Could you check a few things on this model? Use its own coordinates, in mm. A direction names the side the tool comes from. Coordinates: 2 decimals unless noted, no trailing zeros. Order: outer loops, then holes, each group sorted by start corner. A loop starts at its lowest first (then second) coordinate and runs counter-clockwise, first axis right, second up. Notation, with made-up numbers: M 54.5,84 L 82.5,84 A26 cw 82.5,117 Z; hole C 1,-26 d8. An arc over 180 degrees is marked long. Put each result on its own line as item: value. Start each with the question number.
```python
from build123d import *
from build123d.topology import SkipClean

# Parameters (mm, degrees)
CUT_EXTRUDE1_DEPTH      = 13.124356
CUT_EXTRUDE1_DEPTH_BACK = 13.124356
SKETCH4_R               = 3
CUT_EXTRUDE2_DEPTH      = 16.556349
CHAMFER1_SIZE           = 0.4
FILLET1_R               = 5


with BuildPart() as part:
    # Sketch1 → Boss-Revolve (revolve)
    with BuildSketch(Plane.XY):
        with BuildLine():
            Line((-7, 0), (7, 0))
            ThreePointArc((7, 0), (0, 7), (-7, 0))
        make_face()
    revolve(axis=Axis((-13.286843, 0, 0), (1, 0, 0)))

    # Sketch2 → Cut-Extrude1 (cut, two sides: drawn at the far end of the back side and taken through both)
    with SkipClean():  # the faces are left unmerged after this step: merging them gives an invalid solid
        with BuildSketch(Plane(origin=(0, 0, 0), x_dir=(0, 0, -1), z_dir=(1, 0, 0)).offset(-CUT_EXTRUDE1_DEPTH_BACK)):
            with BuildLine():
                Line((-5, 4.898979), (-5, -4.898979))
                ThreePointArc((-5, -4.898979), (-7, 0), (-5, 4.898979))
            make_face()
            with BuildLine():
                Line((5, 4.898979), (5, -4.898979))
                ThreePointArc((5, -4.898979), (7, 0), (5, 4.898979))
            make_face()
        extrude(amount=CUT_EXTRUDE1_DEPTH + CUT_EXTRUDE1_DEPTH_BACK, mode=Mode.SUBTRACT)

    # Sketch4 → Cut-Extrude2 (cut, through all)
    with SkipClean():  # the faces are left unmerged after this step: merging them gives an invalid solid
        with BuildSketch(Plane.XY.offset(5)):
            Circle(SKETCH4_R)
        extrude(amount=-CUT_EXTRUDE2_DEPTH, mode=Mode.SUBTRACT)

    # Sketch5 → Boss-Revolve1 (revolve)
    with SkipClean():  # the faces are left unmerged after this step: merging them gives an invalid solid
        with BuildSketch(Plane.XY, mode=Mode.PRIVATE) as boss_revolve1_sk:
            Polygon((3.469445, 3.45875), (3.469445, 0), (50, 0), (50, 4), (28, 4), (27.062528, 3.45875), align=None)
        revolve(boss_revolve1_sk.sketch.rotate(Axis((0, 0, 0), (1, 0, 0)), 180), axis=Axis((0, 0, 0), (1, 0, 0)))

    # Chamfer1
    chamfer1_edges = [part.edges().sort_by_distance(p)[0] for p in [
        (50, 4, 0),
    ]]
    chamfer(chamfer1_edges, length=CHAMFER1_SIZE)

    # Sketch6 → Cut-Revolve1 (revolve, cut)
    with SkipClean():  # the faces are left unmerged after this step: merging them gives an invalid solid
        with BuildSketch(Plane.XY, mode=Mode.PRIVATE) as cut_revolve1_sk:
            Polygon((49.375018, 4), (50.624982, 4), (50, 2.9175), align=None)
        revolve(cut_revolve1_sk.sketch.rotate(Axis((0, 0, 0), (1, 0, 0)), 180), axis=Axis((0, 0, 0), (1, 0, 0)), mode=Mode.SUBTRACT)

    # Fillet1
    fillet1_edges = [part.edges().sort_by_distance(p)[0] for p in [
        (6.085807, 0, -3.45875),
    ]]
    fillet(fillet1_edges, radius=FILLET1_R)


solid = part.part
```
Item 1: If we section it at A-A on x = 9: Write out the boundary of the cut face in (y, z), then the cut area to 3 significant figures.
Item 2: If we mould it in two halves opening along X, with no side actions, what happens to faces 1 (the flat face through (-0.1, -3.2, -5)), 2 (the flat face through (50, 0, 0)), 3 (the cylindrical face through (17.656, 2.745, 2.105))? For each: released by +X, released by -X, zero draft, split by the parting line, or undercut.
Item 3: For faces 4 (the cylindrical face through (-3, 0, 0)), 5 (the cylindrical face through (38.538, 0.867, 3.905)), which set-ups out of +Z, -Z, +X, -X, +Y, -Y let a thin tool reach every point of the face, with its end or its side?
Item 4: I need wall thicknesses on probe 1 along X at (y, z) = (-0.25, 0.25); probe 2 along Y at (x, z) = (0, -0.25); probe 3 along Y at (x, z) = (39, 0.25). Which ranges of each line are inside material? Lowest first, please.
Item 5: If we section it at B-B on y = -5.75: Write out the boundary of the cut face in (x, z).
Item 6: For pin 1 Ø2 at (x, z) = (28.5, 3) entering from -Y; pin 2 Ø3 at (y, z) = (3, -1.5) entering from -X; pin 3 Ø4 at (x, y) = (30.5, -5) entering from +Z, each with a flat end and sliding along its axis, tell me the tip position at first contact or that it passes through.
Geometry check:
1. outline: C 0,0 d6.92
1. area: 37.6 mm²
2. face 1: zero draft
2. face 2: released by +X
2. face 3: undercut
3. face 4: +Z, -Z
3. face 5: +X
4. probe 1: x = -6.99 to -2.99, 2.99 to 50
4. probe 2: y = -7 to -3, 3 to 7
4. probe 3: y = -3.99 to 3.99
5. outline: C 0,0 d7.98
6. pin 1: stops at y = -3.46
6. pin 2: stops at x = -6.75
6. pin 3: stops at z = 2.65
